Can you work these out from the model? Positions are in its coordinate system, mm. A direction names the side the tool comes from. Give positions to 0.01 mm unless a question says otherwise; leave off trailing zeros. Loops run counter-clockwise (first coordinate to the right, second up) from the corner with the lowest first, then second, coordinate; pieces in that order, holes last. Notation, with made-up numbers: (26.25, 63) - (68.25, 63) arc R26 ccw to (68.25, 95) - close; hole circle Ø2 at (-38, 21.25). An arc over 180 degrees is marked (long way). Answer as a JSON object with one key per item and string values.
```python
from build123d import *

# Parameters (mm, degrees)
SKETCH_1_W          = 30
SKETCH_1_H          = 65
EXTRUDE_1_DEPTH     = 3
CUT_EXTRUDE_1_REACH = 37.92


with BuildPart() as part:
    # 草图1 → 凸台-拉伸1 (new body)
    with BuildSketch(Plane.XY):
        Rectangle(SKETCH_1_W, SKETCH_1_H)
    extrude(amount=EXTRUDE_1_DEPTH)

    # 草图2 → 切除-拉伸1 (cut, up to next)
    with BuildSketch(Plane.XY.offset(3), mode=Mode.PRIVATE) as cut_extrude_1_sk1:
        with BuildLine():
            Line((-11, -26.5), (-11, 8.5))
            ThreePointArc((-11, 8.5), (-8.5, 11), (-6, 8.5))
            Line((-6, 8.5), (-6, -26.5))
            ThreePointArc((-6, -26.5), (-8.5, -29), (-11, -26.5))
        make_face()
    cut_extrude_1_tool1 = extrude(cut_extrude_1_sk1.sketch, amount=-CUT_EXTRUDE_1_REACH, mode=Mode.PRIVATE) & part.part
    cut_extrude_1 = cut_extrude_1_tool1.solids().sort_by_distance((-8.5, -9, 3))[0]
    add(cut_extrude_1, mode=Mode.SUBTRACT)

    # 镜向1: 切除-拉伸1 across plane
    add(cut_extrude_1.mirror(Plane(origin=(0, 0, 0), x_dir=(0, 0, 1), z_dir=(1, 0, 0))), mode=Mode.SUBTRACT)


solid = part.part
```
1) If we mould it in two halves opening along Y, with no side actions, what happens to faces 3 (the flat face through (11, -9, 2)), 4 (the flat face through (0, 0, 3)), 5 (the flat face through (0, 32.5, 1)), 6 (the cylindrical face through (8.6, 11, 1.5))? For each: released by +Y, released by -Y, zero draft, split by the parting line, or undercut.
Check sheet entries:
{"face 3": "undercut", "face 4": "zero draft", "face 5": "released by +Y", "face 6": "undercut"}
2) Imagine slicing it at C-C on x = 8.5. Write out the boundary of the cut face in (y, z).
Check sheet entries:
{"outline": "(-32.5, 0) - (-29, 0) - (-29, 3) - (-32.5, 3) - close; (11, 0) - (32.5, 0) - (32.5, 3) - (11, 3) - close"}
3) Imagine slicing it at B-B on z = 2.1. Write out the boundary of the cut face in (x, y), and give its area (3 significant figures).
Check sheet entries:
{"outline": "(-15, -32.5) - (15, -32.5) - (15, 32.5) - (-15, 32.5) - close; hole (-11, -26.5) arc R2.5 ccw to (-6, -26.5) - (-6, 8.5) arc R2.5 ccw to (-11, 8.5) - close; hole (6, -26.5) arc R2.5 ccw to (11, -26.5) - (11, 8.5) arc R2.5 ccw to (6, 8.5) - close", "area": "1,560 mm2"}
4) Which directions (+Z, -Z, +X, -X, +Y, -Y) give clear straight access to the entire face, cutting with the end or side of a thin tool? Please do faces 1 (the cylindrical face through (-8.6, 11, 1.5)), 2 (the flat face through (-15, 0, 1)).
Check sheet entries:
{"face 1": "+Z, -Z", "face 2": "+Z, -Z, -X, +Y, -Y"}
5) I need wall thicknesses on L1, parallel to X at y = -7, z = 1.9; L2, parallel to X at y = 9, z = 1.8; L3, parallel to Y at x = -8.25, z = 2.55. Which ranges of each line are inside material? Lowest first, please.
Check sheet entries:
{"L1": "-15 to -11, -6 to 6, 11 to 15", "L2": "-15 to -10.95, -6.05 to 6.05, 10.95 to 15", "L3": "-32.5 to -28.99, 10.99 to 32.5"}
6) Imagine slicing it at A-A on y = -19.5. Write out the boundary of the cut face in (x, z), and give its area (3 significant figures).
Check sheet entries:
{"outline": "(-15, 0) - (-11, 0) - (-11, 3) - (-15, 3) - close; (-6, 0) - (6, 0) - (6, 3) - (-6, 3) - close; (11, 0) - (15, 0) - (15, 3) - (11, 3) - close", "area": "60.0 mm2"}
